from build123d import *

# Parameters (mm, degrees)
SKETCH1_W                   = 25
SKETCH1_H                   = 310
BOSS_EXTRUDE1_DEPTH         = 20
SKETCH3_R                   = 4.25
CUT_EXTRUDE1_DEPTH          = 30
SKETCH5_R                   = 6.5
CUT_EXTRUDE3_DEPTH          = 10
M12X1_25_TAPPED_HOLE1_D     = 10.5
M12X1_25_TAPPED_HOLE1_DEPTH = 30.25
M12X1_25_TAPPED_HOLE1_TIP   = 3.15451825


with BuildPart() as part:
    # Sketch1 → Boss-Extrude1 (new body)
    with BuildSketch(Plane.XY):
        Rectangle(SKETCH1_W, SKETCH1_H)
    extrude(amount=BOSS_EXTRUDE1_DEPTH)

    # Sketch3 → Cut-Extrude1 (cut)
    with BuildSketch(Plane.XY.offset(20)):
        with Locations((0, 140)):
            Circle(SKETCH3_R)
        with Locations((0, 45)):
            Circle(SKETCH3_R)
        with Locations((0, -45)):
            Circle(SKETCH3_R)
        with Locations((0, -140)):
            Circle(SKETCH3_R)
    extrude(amount=-CUT_EXTRUDE1_DEPTH, mode=Mode.SUBTRACT)

    # Sketch5 → Cut-Extrude3 (cut)
    with BuildSketch(Plane(origin=(0, 0, 0), x_dir=(-1, 0, 0), z_dir=(0, 0, -1))):
        with Locations((0, 140)):
            Circle(SKETCH5_R)
        with Locations((0, 45)):
            Circle(SKETCH5_R)
        with Locations((0, -45)):
            Circle(SKETCH5_R)
        with Locations((0, -140)):
            Circle(SKETCH5_R)
    extrude(amount=-CUT_EXTRUDE3_DEPTH, mode=Mode.SUBTRACT)

    # M12x1.25 Tapped Hole1
    with Locations(Plane(origin=(0, 0, 0), x_dir=(-1, 0, 0), z_dir=(0, 0, -1))):
        with Locations((0, 90), (0, 0), (0, -90)):
            Hole(M12X1_25_TAPPED_HOLE1_D / 2, depth=M12X1_25_TAPPED_HOLE1_DEPTH)
            with Locations((0, 0, -(M12X1_25_TAPPED_HOLE1_DEPTH + M12X1_25_TAPPED_HOLE1_TIP / 2))):  # 118° drill point
                Cone(0, M12X1_25_TAPPED_HOLE1_D / 2, M12X1_25_TAPPED_HOLE1_TIP, mode=Mode.SUBTRACT)


solid = part.part
The model under review builds one solid part; all positions refer to its coordinate system, in mm. A direction names the side the tool comes from. Round coordinates to 2 decimals unless told otherwise and drop trailing zeros. Order: outer loops, then holes, each group sorted by start corner. A loop starts at its lowest first (then second) coordinate and runs counter-clockwise, first axis right, second up. Notation, with made-up numbers: (57.25, 16.5) - (68.25, 16.5) arc R23 cw to (68.25, 41.5) - close; hole circle Ø11 at (45.25, 81). An arc over 180 degrees is marked (long way). Use one line per item in the form item = value.
Q1. Mouldability with a two-part tool opening along Y and no side actions: class faces 1 (the flat face through (-6, 2, 20)), 2 (the flat face through (-1.4, -49.2, 10)), 3 (the flat face through (0, -155, 10)) as pulls with the +Y half, pulls with the -Y half, needs draft (parallel to the pull), parting line crosses it, or undercut.
Response values:
face_1 = needs draft
face_2 = undercut
face_3 = pulls with the -Y half
Q2. Add section B-B on y = 0. Give the boundary of the cut face in (x, z).
Response values:
outline = (-12.5, 0) - (-5.25, 0) - (-5.25, 20) - (-12.5, 20) - close; (5.25, 0) - (12.5, 0) - (12.5, 20) - (5.25, 20) - close
Q3. Add section D-D on y = -140. Give the boundary of the cut face in (x, z), then the cut area to 3 significant figures.
Response values:
outline = (-12.5, 0) - (-6.5, 0) - (-6.5, 10) - (-4.25, 10) - (-4.25, 20) - (-12.5, 20) - close; (4.25, 10) - (6.5, 10) - (6.5, 0) - (12.5, 0) - (12.5, 20) - (4.25, 20) - close
area = 285 mm^2
Q4. Clearance check with a flat-ended pin moving along its axis: P1, Ø11, axis at x = 0, y = -45, coming from the -Z side. State where the tip first meets the part, or that it passes through.
Response values:
P1 = 10
Q5. Add section A-A on z = 13.5. Give the boundary of the cut face in (x, y), then the cut area to 3 significant figures.
Response values:
outline = (-12.5, -155) - (12.5, -155) - (12.5, 155) - (-12.5, 155) - close; hole circle Ø10.5 at (0, -90); hole circle Ø10.5 at (0, 0); hole circle Ø10.5 at (0, 90); hole circle Ø8.5 at (0, -140); hole circle Ø8.5 at (0, -45); hole circle Ø8.5 at (0, 45); hole circle Ø8.5 at (0, 140)
area = 7,260 mm^2
Q6. Add section C-C on x = 0. Give the number of separate pieces and of enclosed holes in the cut face, then the cut area to 3 significant figures.
Response values:
separate_pieces = 8
enclosed_holes = 0
area = 4,710 mm^2
Q7. Tool access review of faces 4 (the cylindrical face through (1.409, -146.345, 4.93)), 5 (the cylindrical face through (-0.553, -135.786, 15.07)): name each direction out of +Z, -Z, +X, -X, +Y, -Y from which nothing blocks a thin tool from reaching the whole face with its end or side.
Response values:
face_4 = -Z
face_5 = +Z, -Z
Q8. To check wall thickness, follow line 1 (X direction, y = -49, z = 6); line 2 (Z direction, x = 1.5, y = -50.5). State the ranges of each line that lie inside material, in increasing order.
Response values:
line_1 = -12.5 to -5.12, 5.12 to 12.5
line_2 = 10 to 20
